For this review, use the dimensioned drawing (mm, ordinates from the lowest corner) and the shaded views. A direction names the side the tool comes from. Coordinates: 2 decimals unless noted, no trailing zeros. Write each loop counter-clockwise with the first axis right and the second up, starting at its lowest first coordinate (ties: lowest second). Pieces come first, ordered by that corner, then holes. Notation, with made-up numbers: (-33, 82.5) - (25, 82.5) arc R21 cw to (25, 93.5) - close; hole circle Ø8 at (0, 33.25). An arc over 180 degrees is marked (long way). Put each result on its own line as item: value.
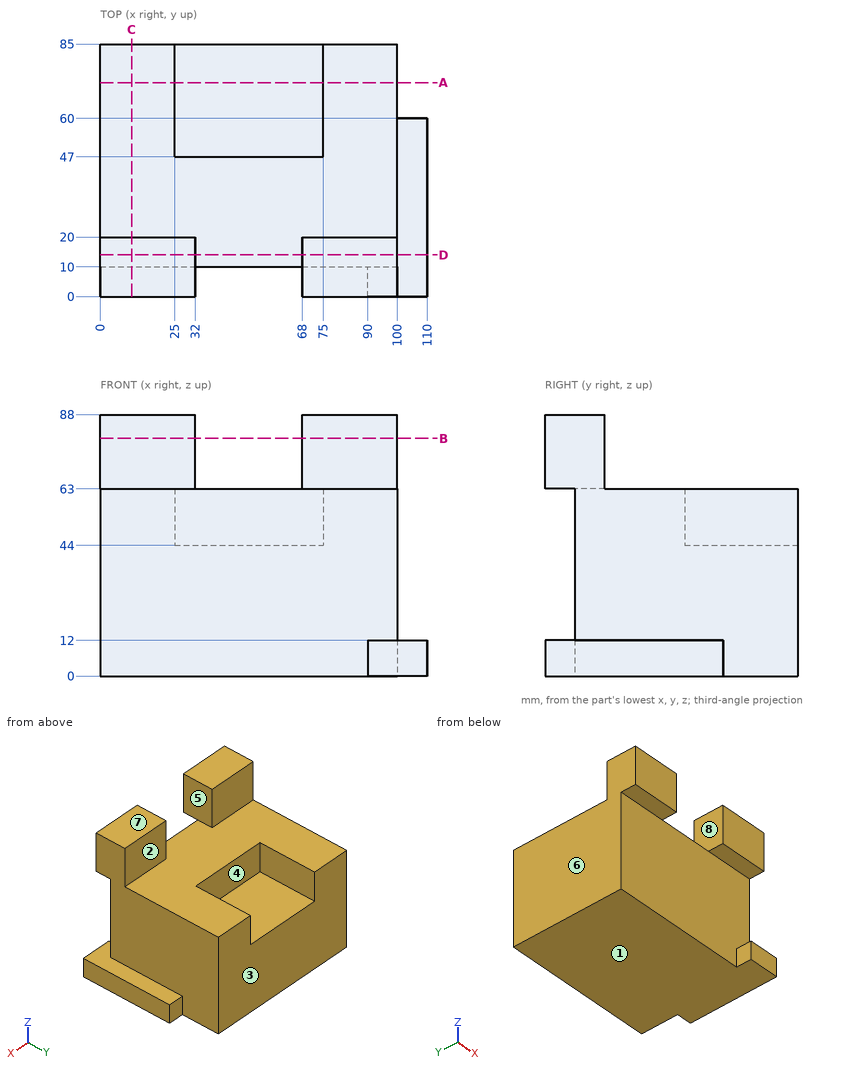
1. Consider section B-B on z = 80. State the section outline as (x, y) points.
Determined:
outline: (0, 0) - (32, 0) - (32, 20) - (0, 20) - close; (68, 0) - (100, 0) - (100, 20) - (68, 20) - close
2. For pin 1 Ø10 at (y, z) = (8, 77) entering from +X; pin 2 Ø12.5 at (x, z) = (20, 70) entering from +Y; pin 3 Ø5 at (x, z) = (105.5, 5) entering from +Y; pin 4 Ø5 at (x, y) = (48, 74.5) entering from -Z, all flat-tipped, find the tip position at first contact; note any pin that passes through.
Determined:
pin 1: stops at x = 100
pin 2: stops at y = 20
pin 3: stops at y = 60
pin 4: stops at z = 0
3. Machinability: for the marked faces 1, 2, 3, 4 and 5, which of the approach directions +Z, -Z, +X, -X, +Y, -Y give a long, thin tool a straight path to every point of the face, cutting with its end or side? Answer none if there is none.
Determined:
face 1: -Z, +X, -X, +Y, -Y
face 2: +Z, +X, -X, +Y
face 3: +Z, -Z, +X, -X, +Y
face 4: +Z, +Y
face 5: +Z, +Y, -Y
4. To check wall thickness, follow probe 1 along X at (y, z) = (72, 46); probe 2 along Y at (x, z) = (97, 81); probe 3 along Z at (x, y) = (39, 53). State the ranges of each line that lie inside material, in increasing order.
Determined:
probe 1: x = 0 to 25, 75 to 100
probe 2: y = 0 to 20
probe 3: z = 0 to 44
5. Consider section A-A on y = 72. State the section outline as (x, z) points, plus the area to 3 significant figures.
Determined:
outline: (0, 0) - (100, 0) - (100, 63) - (75, 63) - (75, 44) - (25, 44) - (25, 63) - (0, 63) - close
area: 5,350 mm^2
6. The part is to be moulded in two halves that separate along X. For the marked faces 6, 7 and 8, say which applies: +X half, -X half, draft (parallel to the pull), parting line (faces both ways), or undercut.
Determined:
face 6: -X half
face 7: draft
face 8: undercut
7. Consider section D-D on y = 14. State the section outline as (x, z) points.
Determined:
outline: (0, 0) - (110, 0) - (110, 12) - (100, 12) - (100, 88) - (68, 88) - (68, 63) - (32, 63) - (32, 88) - (0, 88) - close
8. Consider section C-C on x = 10.5. State the section outline as (y, z) points, plus the area to 4 significant figures.
Determined:
outline: (0, 63) - (10, 63) - (10, 0) - (85, 0) - (85, 63) - (20, 63) - (20, 88) - (0, 88) - close
area: 5,225 mm^2
